The listing builds one solid part. Answer for the finished solid, in the listing's coordinates (mm). Face numbers are marked on the shaded views. A direction names the side the tool comes from. Coordinates: 2 decimals unless noted, no trailing zeros. Write each loop counter-clockwise with the first axis right and the second up, starting at its lowest first coordinate (ties: lowest second). Pieces come first, ordered by that corner, then holes.
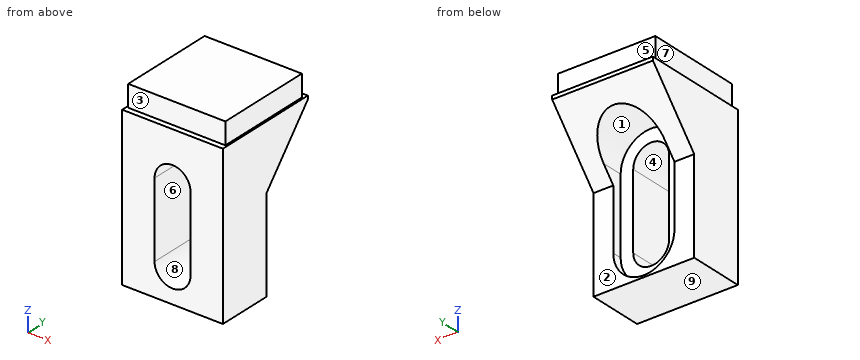
from build123d import *

# Parameters (mm, degrees)
SKETCH1_W               = 13.5
SKETCH1_H               = 13.5
BOSS_EXTRUDE1_DEPTH     = 1.5
SKETCH2_W               = 14
SKETCH2_H               = 15
BOSS_EXTRUDE2_DEPTH     = 22
CUT_EXTRUDE2_DEPTH      = 29.363709207
CUT_EXTRUDE2_DEPTH_BACK = 29.363709207
CUT_EXTRUDE3_DEPTH      = 8.6
CUT_EXTRUDE4_DEPTH      = 11.3


with BuildPart() as part:
    # Sketch1 → Boss-Extrude1 (new, symmetric)
    with BuildSketch(Plane.XY):
        Rectangle(SKETCH1_W, SKETCH1_H)
    extrude(amount=BOSS_EXTRUDE1_DEPTH, both=True)

    # Sketch2 → Boss-Extrude2 (add)
    with BuildSketch(Plane(origin=(0, 0, -1.5), x_dir=(-1, 0, 0), z_dir=(0, 0, -1))):
        Rectangle(SKETCH2_W, SKETCH2_H)
    extrude(amount=BOSS_EXTRUDE2_DEPTH)

    # Sketch3 → Cut-Extrude2 (cut, two sides: drawn at the far end of the back side and taken through both)
    with BuildSketch(Plane(origin=(7, 0, 0), x_dir=(0, 0, -1), z_dir=(1, 0, 0)).offset(-CUT_EXTRUDE2_DEPTH_BACK)):
        Polygon((85.930906916, 0.2), (23.5, 0.2), (10.5, 0.2), (2, 7.5), (-45.361724521, 48.175363412), (-2.507621852, 165.452805564), (128.785009585, 117.477442152), align=None)
    extrude(amount=CUT_EXTRUDE2_DEPTH + CUT_EXTRUDE2_DEPTH_BACK, mode=Mode.SUBTRACT)

    # Sketch5 → Cut-Extrude3 (cut)
    with BuildSketch(Plane(origin=(0, 7.5, 0), x_dir=(1, 0, 0), z_dir=(0, 1, 0))):
        with BuildLine():
            Line((-4.25, 19), (-4.25, 8.5))
            ThreePointArc((-4.25, 8.5), (0, 4.25), (4.25, 8.5))
            Line((4.25, 8.5), (4.25, 19))
            ThreePointArc((4.25, 19), (0, 23.25), (-4.25, 19))
        make_face()
    extrude(amount=-CUT_EXTRUDE3_DEPTH, mode=Mode.SUBTRACT)

    # Sketch4 → Cut-Extrude4 (cut)
    with BuildSketch(Plane(origin=(0, 0.2, 0), x_dir=(1, 0, 0), z_dir=(0, 1, 0))):
        with BuildLine():
            Line((2.5, 19), (2.5, 8.5))
            ThreePointArc((2.5, 8.5), (0, 6), (-2.5, 8.5))
            Line((-2.5, 8.5), (-2.5, 19))
            ThreePointArc((-2.5, 19), (0, 21.5), (2.5, 19))
        make_face()
    extrude(amount=-CUT_EXTRUDE4_DEPTH, mode=Mode.SUBTRACT)


solid = part.part
Q1. Which of the six approach directions +Z, -Z, +X, -X, +Y, -Y give full straight-line access (tool end or side, diameter ignored) to the marked faces 1, 2, 3, 4 and 5?
Answers below:
face 1: +Y
face 2: -Z, +X, -X, +Y
face 3: +Z, +X, -X, -Y
face 4: +Y, -Y
face 5: +Z, +X, -X, +Y
Q2. Determine the mould class of the marked faces 6, 7, 8 and 9 for opening direction X: released by +X, released by -X, zero draft, split by the parting line, or undercut.
Answers below:
face 6: undercut
face 7: released by -X
face 8: undercut
face 9: zero draft
Q3. Find the intervals of material crossed by probe 1 along X at (y, z) = (-1.5, -14.25); probe 2 along X at (y, z) = (-0.75, -11); probe 3 along X at (y, z) = (0.5, 0.75), in increasing order.
Answers below:
probe 1: x = -7 to -2.5, 2.5 to 7
probe 2: x = -7 to -4.25, 4.25 to 7
probe 3: x = -6.75 to 6.75
Q4. Given pin 1 (1.5 mm diameter, centred on y = -0.5, z = -0.5, fed in from +X); pin 2 (3.5 mm diameter, centred on x = -2, z = 0.5, fed in from -Y); pin 3 (4 mm diameter, centred on x = -3, z = -19, fed in from +Y), each flat-ended and moving along its own axis, determine where each tip first touches the part or whether it passes through.
Answers below:
pin 1: stops at x = 6.75
pin 2: stops at y = -6.75
pin 3: stops at y = 0.2
Q5. The part is cut by section D-D, the plane x = -1.75. Write down the section's boundary in (y, z), then the cut area to 3 significant figures.
Answers below:
outline: (-7.5, -23.5) - (0.2, -23.5) - (0.2, -22.87) - (-1.1, -22.87) - (-1.1, -20.79) - (-7.5, -20.79) - close; (-7.5, -6.71) - (-1.1, -6.71) - (-1.1, -4.63) - (5.24, -4.63) - (7.5, -2) - (7.5, -1.5) - (6.75, -1.5) - (6.75, 1.5) - (-6.75, 1.5) - (-6.75, -1.5) - (-7.5, -1.5) - close
area: 116 mm2
Q6. The part is cut by section C-C, the plane x = 5.5. Write down the section's boundary in (y, z).
Answers below:
outline: (-7.5, -23.5) - (0.2, -23.5) - (0.2, -10.5) - (7.5, -2) - (7.5, -1.5) - (6.75, -1.5) - (6.75, 1.5) - (-6.75, 1.5) - (-6.75, -1.5) - (-7.5, -1.5) - close
Q7. The part is cut by section B-B, the plane z = -11. Write down the section's boundary in (x, y), then the cut area to 4 significant figures.
Answers below:
outline: (-7, -7.5) - (-2.5, -7.5) - (-2.5, -1.1) - (-4.25, -1.1) - (-4.25, 0.2) - (-7, 0.2) - close; (2.5, -7.5) - (7, -7.5) - (7, 0.2) - (4.25, 0.2) - (4.25, -1.1) - (2.5, -1.1) - close
area: 64.75 mm2
Q8. The part is cut by section A-A, the plane y = -0.75. Write down the section's boundary in (x, z), then the cut area to 3 significant figures.
Answers below:
outline: (-7, -23.5) - (7, -23.5) - (7, -1.5) - (6.75, -1.5) - (6.75, 1.5) - (-6.75, 1.5) - (-6.75, -1.5) - (-7, -1.5) - close; hole (-4.25, -19) arc R4.25 ccw to (4.25, -19) - (4.25, -8.5) arc R4.25 ccw to (-4.25, -8.5) - close
area: 203 mm2
